Design review of the part built by this model. Coordinates are the model's own, in mm. A direction names the side the tool comes from. Give positions to 0.01 mm unless a question says otherwise; leave off trailing zeros. Loops run counter-clockwise (first coordinate to the right, second up) from the corner with the lowest first, then second, coordinate; pieces in that order, holes last. Notation, with made-up numbers: M -36.5,60.25 L 9.5,60.25 A28 ccw 9.5,83.25 Z; hole C -9,-27.5 d3. An arc over 180 degrees is marked long. Use a Markdown table: item, result. Add a question column.
(1) Insertion check: pin 1 Ø1 at (x, y) = (11.5, 0.5) entering from +Z; pin 2 Ø1 at (x, y) = (0, -8) entering from -Z; pin 3 Ø1.5 at (x, z) = (0, 9.5) entering from -Y. Each pin has a flat end and moves straight along its axis. Give the tip position at first contact, or say it passes through.
(2) Add section C-C, the plane x = 0.5. Give the boundary of the cut face in (y, z), then the cut area to 3 significant figures.
(3) Add section D-D, the plane y = 5. Give the boundary of the cut face in (x, z), then the cut area to 3 significant figures.
(4) Add section A-A, the plane y = 0. Give the boundary of the cut face in (x, z).
(5) For probe 1 along Y at (x, z) = (0, 1.5); probe 2 along Y at (x, z) = (0, 4.25); probe 3 along Z at (x, y) = (6.5, 14), list the stretches that pass through material, from the lowest coordinate up.
(6) Add section B-B, the plane x = -10. Give the boundary of the cut face in (y, z).
(7) For faces 1 (the face through (0.479, 3.998, 8.345)), 2 (the face through (3, 0, 0)), 3 (the face through (-1.409, -6.345, 7.437)), list the 3-axis set-ups (+Z, -Z, +X, -X, +Y, -Y) from which the entire face can be reached by the end or side of a thin tool; tool diameter is ignored.
(8) Draft analysis for pull direction Y (two halves, no side actions). For faces 4 (the face through (-9.24, -6.48, 1.52)), 5 (the face through (-3.47, -15.62, 1.48)), 6 (the face through (1, 2, 12)), 7 (the face through (-0.16, 13.24, 1.52)), state which applies: pulls with the +Y half, pulls with the -Y half, needs draft (parallel to the pull), parting line crosses it, or undercut.
```python
from build123d import *

# Parameters (mm, degrees)
SKETCH1_R             = 16
BOSS_EXTRUDE1_DEPTH   = 3
SKETCH2_R             = 6.5
BOSS_EXTRUDE2_DEPTH   = 9
SKETCH3_R             = 2
CUT_EXTRUDE1_DEPTH    = 22
SKETCH4_R             = 1
CUT_EXTRUDE2_DEPTH    = 10
M3_TAPPED_HOLE6_D     = 2.5
M3_TAPPED_HOLE6_DEPTH = 12


with BuildPart() as part:
    # Sketch1 → Boss-Extrude1 (new body)
    with BuildSketch(Plane.XY):
        Circle(SKETCH1_R)
    extrude(amount=BOSS_EXTRUDE1_DEPTH)

    # Sketch2 → Boss-Extrude2 (add)
    with BuildSketch(Plane.XY.offset(3)):
        Circle(SKETCH2_R)
    extrude(amount=BOSS_EXTRUDE2_DEPTH)

    # Sketch3 → Cut-Extrude1 (cut)
    with BuildSketch(Plane(origin=(0, 0, 0), x_dir=(-1, 0, 0), z_dir=(0, 0, -1))):
        Circle(SKETCH3_R)
    extrude(amount=-CUT_EXTRUDE1_DEPTH, mode=Mode.SUBTRACT)

    # Sketch16 → M3 Tapped Hole5 (revolve, cut)
    with BuildSketch(Plane(origin=(0, 0, 9.5), x_dir=(0, 0, -1), z_dir=(1, 0, 0))):
        Polygon((0, 0), (0, 8.251075774), (1.25, 7.5), (1.25, 0), align=None)
    revolve(axis=Axis((0, -6.35, 9.5), (0, 1, 0)), mode=Mode.SUBTRACT)

    # Sketch4 → Cut-Extrude2 (cut)
    with BuildSketch(Plane(origin=(0, 0, 0), x_dir=(-1, 0, 0), z_dir=(0, 0, -1))):
        with Locations((0, 12)):
            Circle(SKETCH4_R)
        with Locations((10.392304845, -6)):
            Circle(SKETCH4_R)
        with Locations((-10.392304845, -6)):
            Circle(SKETCH4_R)
    extrude(amount=-CUT_EXTRUDE2_DEPTH, mode=Mode.SUBTRACT)

    # M3 Tapped Hole6
    with Locations(Plane(origin=(0, 0, 0), x_dir=(-1, 0, 0), z_dir=(0, 0, -1))):
        with Locations((0, 12), (-10.392304845, -6), (10.392304845, -6)):
            Hole(M3_TAPPED_HOLE6_D / 2, depth=M3_TAPPED_HOLE6_DEPTH)


solid = part.part
```
Established:
| question | item | result |
|---|---|---|
| 1 | pin 1 | z = 3 |
| 1 | pin 2 | z = 0 |
| 1 | pin 3 | y = -6.5 |
| 2 | outline | M -15.99,0 L -1.94,0 L -1.94,12 L -6.48,12 L -6.48,3 L -15.99,3 Z; M 1.94,0 L 10.85,0 L 10.85,3 L 6.48,3 L 6.48,8.35 L 1.94,8.35 Z; M 1.94,10.65 L 6.48,10.65 L 6.48,12 L 1.94,12 Z; M 13.15,0 L 15.99,0 L 15.99,3 L 13.15,3 Z |
| 2 | area | 149 mm^2 |
| 3 | outline | M -15.2,0 L 15.2,0 L 15.2,3 L 4.15,3 L 4.15,12 L -4.15,12 L -4.15,3 L -15.2,3 Z; hole C 0,9.5 d2.5 |
| 3 | area | 161 mm^2 |
| 4 | outline | M -16,0 L -2,0 L -2,12 L -6.5,12 L -6.5,3 L -16,3 Z; M 2,0 L 16,0 L 16,3 L 6.5,3 L 6.5,12 L 2,12 Z |
| 5 | probe 1 | -16 to -2, 2 to 10.75, 13.25 to 16 |
| 5 | probe 2 | -6.5 to -2, 2 to 6.5 |
| 5 | probe 3 | 0 to 3 |
| 6 | outline | M -12.49,0 L -7.19,0 L -7.19,3 L -12.49,3 Z; M -4.81,0 L 12.49,0 L 12.49,3 L -4.81,3 Z |
| 7 | face 1 | +Y |
| 7 | face 2 | -Z, +X, -X, +Y, -Y |
| 7 | face 3 | +Z |
| 8 | face 4 | undercut |
| 8 | face 5 | parting line crosses it |
| 8 | face 6 | needs draft |
| 8 | face 7 | undercut |
